Design review of the part built by this model. Coordinates are the model's own, in mm. Face numbers are marked on the shaded views. A direction names the side the tool comes from. Coordinates: 2 decimals unless noted, no trailing zeros. Write each loop counter-clockwise with the first axis right and the second up, starting at its lowest first coordinate (ties: lowest second). Pieces come first, ordered by that corner, then holes.
Q1. Machinability: for the marked faces 1, 2 and 3, which of the approach directions +Z, -Z, +X, -X, +Y, -Y give a long, thin tool a straight path to every point of the face, cutting with its end or side? Answer none if there is none.
Q2. Take a section at A-A (z = 25). Give the boundary of the cut face in (x, y).
Q3. Mouldability with a two-part tool opening along X and no side actions: class the marked faces 4, 5 and 6 as pulls with the +X half, pulls with the -X half, needs draft (parallel to the pull), parting line crosses it, or undercut.
Q4. Take a section at C-C (z = 56). Give the boundary of the cut face in (x, y), and give its area (3 significant figures).
Q5. Insertion check: pin 1 (1 mm diameter, centred on y = 13, z = 65, fed in from -X); pin 2 (1 mm diameter, centred on x = 4.5, z = 24.5, fed in from +Y); pin 3 (12 mm diameter, centred on x = 73, z = 16.5, fed in from +Y); pin 4 (11 mm diameter, centred on y = 29, z = 62, fed in from -X). Each pin has a flat end and moves straight along its axis. Give the tip position at first contact, or say it passes through.
Q6. Take a section at D-D (x = 28). Give the boundary of the cut face in (y, z).
Q7. Take a section at B-B (y = -37). Give the boundary of the cut face in (x, z), and give its area (3 significant figures).
Q8. For probe 1 along Y at (x, z) = (93, 62); probe 2 along X at (y, z) = (-24.5, 74); probe 3 along Z at (x, y) = (75.5, 31.5), list the stretches that pass through material, from the lowest coordinate up.
```python
from build123d import *

# Parameters (mm, degrees)
ARM_PLATE_SKETCH_R        = 9
ARM_PLATE_SKETCH_R_2      = 14
ARM_PLATE_DEPTH           = 9
MOUNTING_FLANGE_SKETCH_R  = 9
MOUNTING_FLANGE_DEPTH     = 18
CONNECTING_BLOCK_SKETCH_W = 9
CONNECTING_BLOCK_SKETCH_H = 94
CONNECTING_BLOCK_DEPTH    = 18
HUB_BOSS_SKETCH_R         = 25
HUB_BOSS_SKETCH_R_2       = 14
HUB_BOSS_DEPTH            = 20
SUPPORT_RIB_DEPTH         = 71
PROFILE_TRIM_CUT_DEPTH    = 143.618371888
FLANGE_CUT_SKETCH_W       = 18
FLANGE_CUT_SKETCH_H       = 2
FLANGE_CUT_DEPTH          = 137.667479724


with BuildPart() as part:
    # Arm Plate Sketch → Arm Plate (new body)
    with BuildSketch(Plane.XY):
        with BuildLine():
            Line((76, 35), (0, 35))
            Line((0, 35), (-78, 18))
            ThreePointArc((-78, 18), (-96, 0), (-78, -18))
            Line((-78, -18), (0, -35))
            Line((0, -35), (76, -35))
            ThreePointArc((76, -35), (84.485281374, -38.514718626), (88, -47))
            Line((88, -47), (88, 47))
            ThreePointArc((88, 47), (84.485281374, 38.514718626), (76, 35))
        make_face()
        with Locations((-78, 0)):
            Circle(ARM_PLATE_SKETCH_R, mode=Mode.SUBTRACT)
        Circle(ARM_PLATE_SKETCH_R_2, mode=Mode.SUBTRACT)
    extrude(amount=ARM_PLATE_DEPTH)



with BuildPart() as body_2:
    # Mounting Flange Sketch → Mounting Flange (new body)
    with BuildSketch(Plane(origin=(88, 0, 0), x_dir=(0, 0, -1), z_dir=(1, 0, 0))):
        with BuildLine():
            Line((-9, 47), (-62, 47))
            ThreePointArc((-62, 47), (-74.727922061, 41.727922061), (-80, 29))
            Line((-80, 29), (-80, -31))
            ThreePointArc((-80, -31), (-74.727922061, -43.727922061), (-62, -49))
            Line((-62, -49), (-9, -49))
            Line((-9, -49), (-9, 47))
        make_face()
        with Locations((-62, 29)):
            Circle(MOUNTING_FLANGE_SKETCH_R, mode=Mode.SUBTRACT)
        with Locations((-62, -31)):
            Circle(MOUNTING_FLANGE_SKETCH_R, mode=Mode.SUBTRACT)
    extrude(amount=MOUNTING_FLANGE_DEPTH)


with BuildPart() as part_1:
    add(part.part)

    add(body_2.part)  # Connecting Block merges body 2
    # Connecting Block Sketch → Connecting Block (add)
    with BuildSketch(Plane(origin=(88, 0, 0), x_dir=(0, 0, -1), z_dir=(1, 0, 0))):
        with Locations((-4.5, 0)):
            Rectangle(CONNECTING_BLOCK_SKETCH_W, CONNECTING_BLOCK_SKETCH_H)
    extrude(amount=CONNECTING_BLOCK_DEPTH)

    # Hub Boss Sketch → Hub Boss (add)
    with BuildSketch(Plane.XY.offset(9)):
        Circle(HUB_BOSS_SKETCH_R)
        Circle(HUB_BOSS_SKETCH_R_2, mode=Mode.SUBTRACT)
    extrude(amount=HUB_BOSS_DEPTH)

    # Support Rib Sketch → Support Rib (add)
    with BuildSketch(Plane.XY.offset(9)):
        with BuildLine():
            Line((88, 0), (88, 5))
            Line((88, 5), (24.494897428, 5))
            ThreePointArc((24.494897428, 5), (24.873403825, 2.51272405), (25, 0))
            ThreePointArc((25, 0), (24.873403825, -2.51272405), (24.494897428, -5))
            Line((24.494897428, -5), (88, -5))
            Line((88, -5), (88, 0))
        make_face()
    extrude(amount=SUPPORT_RIB_DEPTH)

    # Profile Trim Cut Sketch → Profile Trim Cut (cut, through all)
    with BuildSketch(Plane.XZ.offset(5)):
        with BuildLine():
            Line((88, 80), (24.494897428, 80))
            Line((24.494897428, 80), (24.494897428, 29))
            ThreePointArc((24.494897428, 29), (62.058045644, 47.264655803), (88, 80))
        make_face()
    extrude(amount=-PROFILE_TRIM_CUT_DEPTH, mode=Mode.SUBTRACT)

    # Flange Cut Sketch → Flange Cut (cut, through all)
    with BuildSketch(Plane(origin=(0, 0, 9), x_dir=(-1, 0, 0), z_dir=(0, 0, -1))):
        with Locations((-97, -48)):
            Rectangle(FLANGE_CUT_SKETCH_W, FLANGE_CUT_SKETCH_H)
    extrude(amount=-FLANGE_CUT_DEPTH, mode=Mode.SUBTRACT)


solid = part_1.part
```
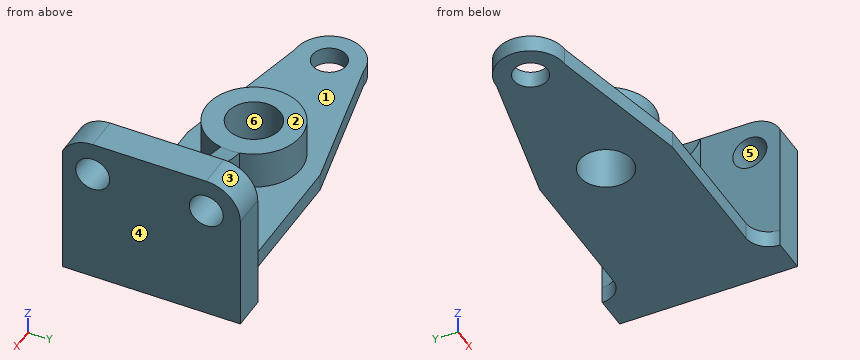
Response:
1. face 1: +Z
1. face 2: +Z, -X, +Y, -Y
1. face 3: +Z, +X, -X, +Y
2. outline: (24.49, -5) - (88, -5) - (88, -47) - (106, -47) - (106, 47) - (88, 47) - (88, 5) - (24.49, 5) arc R25 ccw (long way) to start; hole circle Ø28 at (0, 0)
3. face 4: pulls with the +X half
3. face 5: needs draft
3. face 6: undercut
4. outline: (71.53, -5) - (88, -5) - (88, -24.29) - (106, -24.29) - (106, 22.29) - (88, 22.29) - (88, 5) - (71.53, 5) - close; (88, -47) - (106, -47) - (106, -37.71) - (88, -37.71) - close; (88, 35.71) - (106, 35.71) - (106, 47) - (88, 47) - close
4. area: 1,370 mm2
5. pin 1: stops at x = 88
5. pin 2: stops at y = 24.68
5. pin 3: stops at y = 5
5. pin 4: passes through
6. outline: (-35, 0) - (35, 0) - (35, 9) - (5, 9) - (5, 29.89) - (-5, 29.89) - (-5, 9) - (-35, 9) - close
7. outline: (82.63, 0) - (106, 0) - (106, 55.29) - (88, 55.29) - (88, 9) - (82.63, 9) - close; (88, 68.71) - (106, 68.71) - (106, 78.97) - (88, 78.97) - close
7. area: 1,230 mm2
8. probe 1: y = -47 to -40, -22 to 20, 38 to 47
8. probe 2: x = 88 to 106
8. probe 3: z = 0 to 9
